```python
from build123d import *

# Parameters (mm, degrees)
HUB_SKETCH_R                = 50
HUB_SKETCH_R_2              = 25
HUB_100_BORE_50_DEPTH       = 60
LEVER_ARM_SKETCH_R          = 9
LEVER_ARM_DEPTH             = 15
ARM_LIGHTENING_WINDOW_DEPTH = 179.185296812
EAR_A_SKETCH_R              = 7.5
MOUNTING_EAR_A_DEPTH        = 22.5
MOUNTING_START              = -22.5
EAR_B_SKETCH_R              = 7.5
MOUNTING_EAR_B_DEPTH        = 22.5
ARM_WEB_SKETCH_R            = 7.5
ARM_WEB_10MM_DEPTH          = 10


with BuildPart() as part:
    # Hub Sketch → Hub Ø100 Bore Ø50 (new body)
    with BuildSketch(Plane(origin=(0, 0, 0), x_dir=(1, 0, 0), z_dir=(0, 1, 0))):
        with Locations(Location((0, 0, 0), (0, 0, 270))):
            Circle(HUB_SKETCH_R)
        with Locations(Location((0, 0, 0), (0, 0, 270))):
            Circle(HUB_SKETCH_R_2, mode=Mode.SUBTRACT)
    extrude(amount=HUB_100_BORE_50_DEPTH)

    # Lever Arm Sketch → Lever Arm (add, symmetric)
    with BuildSketch(Plane(origin=(0, 30, 0), x_dir=(1, 0, 0), z_dir=(0, 1, 0))):
        with BuildLine():
            Line((11.808098134, 48.585685325), (150, 15))
            ThreePointArc((150, 15), (165, 0), (150, -15))
            Line((150, -15), (11.808098134, -48.585685325))
            ThreePointArc((11.808098134, -48.585685325), (50, 0), (11.808098134, 48.585685325))
        make_face()
        with Locations(Location((150, 0, 0), (0, 0, 270))):
            Circle(LEVER_ARM_SKETCH_R, mode=Mode.SUBTRACT)
    extrude(amount=LEVER_ARM_DEPTH, both=True)

    # Arm Window Sketch → Arm Lightening Window (cut, through all)
    with BuildSketch(Plane(origin=(0, 45, 0), x_dir=(1, 0, 0), z_dir=(0, 1, 0))):
        with BuildLine():
            Line((127.366472028, 10.209677932), (70.90304943, 23.932354284))
            ThreePointArc((70.90304943, 23.932354284), (61.591288857, 21.405178334), (58.749796974, 12.184471902))
            ThreePointArc((58.749796974, 12.184471902), (60, 0), (58.749796974, -12.184471902))
            ThreePointArc((58.749796974, -12.184471902), (61.591288857, -21.405178334), (70.90304943, -23.932354284))
            Line((70.90304943, -23.932354284), (127.366472028, -10.209677932))
            ThreePointArc((127.366472028, -10.209677932), (132.927164163, -6.594751643), (135.002911441, -0.29552452))
            ThreePointArc((135.002911441, -0.29552452), (135, 0), (135.002911441, 0.29552452))
            ThreePointArc((135.002911441, 0.29552452), (132.927164163, 6.594751643), (127.366472028, 10.209677932))
        make_face()
    extrude(amount=-ARM_LIGHTENING_WINDOW_DEPTH, mode=Mode.SUBTRACT)

    # Ear A Sketch → Mounting Ear A (add)
    with BuildSketch(Plane(origin=(0, 60, 0), x_dir=(1, 0, 0), z_dir=(0, 1, 0))):
        with BuildLine():
            Line((-48.770060726, -10.836899613), (-68.121778265, -22.009618943))
            ThreePointArc((-68.121778265, -22.009618943), (-73.612159322, -42.5), (-53.121778265, -47.990381057))
            Line((-53.121778265, -47.990381057), (-33.644953635, -36.745431114))
            ThreePointArc((-33.644953635, -36.745431114), (-43.203476292, -24.956389512), (-48.770060726, -10.836899613))
        make_face()
        with Locations(Location((-60.621778265, -35, 0), (0, 0, 270))):
            Circle(EAR_A_SKETCH_R, mode=Mode.SUBTRACT)
    extrude(amount=-MOUNTING_EAR_A_DEPTH)

    # Ear B Sketch → Mounting Ear B (add)
    with BuildSketch(Plane(origin=(0, 60, 0), x_dir=(1, 0, 0), z_dir=(0, 1, 0)).offset(MOUNTING_START)):
        with BuildLine():
            Line((-33.806779105, 36.838861092), (-53.121778265, 47.990381057))
            ThreePointArc((-53.121778265, 47.990381057), (-73.612159322, 42.5), (-68.121778265, 22.009618943))
            Line((-68.121778265, 22.009618943), (-48.806779105, 10.858098979))
            ThreePointArc((-48.806779105, 10.858098979), (-43.301270189, 25), (-33.806779105, 36.838861092))
        make_face()
        with Locations(Location((-60.621778265, 35, 0), (0, 0, 270))):
            Circle(EAR_B_SKETCH_R, mode=Mode.SUBTRACT)
    extrude(amount=MOUNTING_EAR_B_DEPTH)

    # Arm Web Sketch → Arm Web 10mm (add)
    with BuildSketch(Plane(origin=(0, 0, 0), x_dir=(1, 0, 0), z_dir=(0, 1, 0))):
        with BuildLine():
            Line((-80, 15), (-50.661233673, 15))
            Line((-50.661233673, 15), (-43.043702026, 15))
            Line((-43.043702026, 15), (-43.043702026, -15))
            Line((-43.043702026, -15), (-80, -15))
            ThreePointArc((-80, -15), (-95, 0), (-80, 15))
        make_face()
        with Locations(Location((-80, 0, 0), (0, 0, 270))):
            Circle(ARM_WEB_SKETCH_R, mode=Mode.SUBTRACT)
    extrude(amount=ARM_WEB_10MM_DEPTH)


solid = part.part
```
The listing builds one solid part. Answer for the finished solid, in the listing's coordinates (mm). A direction names the side the tool comes from. Round coordinates to 2 decimals unless told otherwise and drop trailing zeros. Loops run counter-clockwise (first coordinate to the right, second up) from the corner with the lowest first, then second, coordinate; pieces in that order, holes last.
Q1. Given pin 1 Ø3 at (x, y) = (-68.5, 6) entering from +Z; pin 2 Ø1 at (y, z) = (12, -5) entering from -X; pin 3 Ø12 at (x, y) = (102.5, 47) entering from +Z; pin 4 Ø13.5 at (x, z) = (-60.62, 35) entering from -Y, each flat-ended and moving along its own axis, determine where each tip first touches the part or whether it passes through.
Q2. Section A-A, the plane x = 0 is taken. Determine the outline of the cut face in (y, z).
Q3. For a pull along X with two mould halves and no side action, classify faces 4 (the face through (60, 30, 0)), 5 (the face through (165, 30, 0)), 6 (the face through (-64, 5, 15)) as released by +X, released by -X, zero draft, split by the parting line, or undercut.
Q4. Section D-D, the plane x = 53 is taken. Determine the outline of the cut face in (y, z), then the cut area to 3 significant figures.
Q5. Find the intervals of material crossed by line 1 (X direction, y = 25.5, z = 0); line 2 (X direction, y = 39, z = 3.5); line 3 (X direction, y = 56, z = -37.5), in increasing order.
Q6. Which of the six approach directions +Z, -Z, +X, -X, +Y, -Y give full straight-line access (tool end or side, diameter ignored) to faces 1 (the face through (-58.329, 48.908, 16.356)), 2 (the face through (98.74, 30.21, 17.167)), 3 (the face through (79.937, 30.21, -32.028))?
Q7. Section B-B, the plane y = 20.5 is taken. Determine the outline of the cut face in (x, z).
Q8. Section C-C, the plane z = -32.5 is taken. Determine the outline of the cut face in (x, y).
Completed:
1. pin 1: stops at z = 15
1. pin 2: stops at x = -49.8
1. pin 3: stops at z = 27.92
1. pin 4: passes through
2. outline: (0, -50) - (60, -50) - (60, -25) - (0, -25) - close; (0, 25) - (60, 25) - (60, 50) - (0, 50) - close
3. face 4: undercut
3. face 5: released by +X
3. face 6: zero draft
4. outline: (15, -38.57) - (45, -38.57) - (45, 38.57) - (15, 38.57) - close
4. area: 2,310 mm2
5. line 1: x = -50 to -25, 25 to 60, 135 to 141, 159 to 165
5. line 2: x = -49.88 to -24.75, 24.75 to 59.9, 134.54 to 141.71, 158.29 to 164.59
5. line 3: x = -75.41 to -67.69, -53.55 to -34.95, -33.07 to 33.07
6. face 1: -X, +Y
6. face 2: +Y, -Y
6. face 3: -Z, +X, +Y, -Y
7. outline: (11.81, -48.59) - (150, -15) arc R15 ccw to (150, 15) - (11.81, 48.59) arc R50 ccw (long way) to start; hole circle Ø50 at (0, 0); hole (58.75, -12.18) arc R10 ccw to (70.9, -23.93) - (127.37, -10.21) arc R10 ccw to (135, -0.3) arc R15 cw to (135, 0.3) arc R10 ccw to (127.37, 10.21) - (70.9, 23.93) arc R10 ccw to (58.75, 12.18) arc R60 cw to start; hole circle Ø18 at (150, 0)
8. outline: (-75.41, 37.5) - (-67.69, 37.5) - (-67.69, 60) - (-75.41, 60) - close; (-53.55, 37.5) - (-38, 37.5) - (-38, 0) - (38, 0) - (38, 15) - (77.99, 15) - (77.99, 45) - (38, 45) - (38, 60) - (-53.55, 60) - close
